Here's the drawing with two shaded views (mm, measured from the low corner). I have some questions. Give positions to 0.01 mm unless a question says otherwise; leave off trailing zeros. Loops run counter-clockwise (first coordinate to the right, second up) from the corner with the lowest first, then second, coordinate; pieces in that order, holes last. Notation, with made-up numbers: (-39.5, -38) -> (-19.5, -38) arc R18 cw to (-19.5, -16) -> close; hole circle Ø11 at (-30, -30). An arc over 180 degrees is marked (long way). Write each question's results on one line, items separated by ' | '. Start each with the question number.
Q1. If we section it at C-C, the plane y = 7.5: Give the number of separate pieces and of enclosed holes in the cut face, plus the area to 3 significant figures.
Q2. Will this pin go through, and if not, where does the flat tip stop? P1, Ø19, axis at x = 21, z = 35, coming from the +Y side.
Q3. If I drill on line 1 along X through (y, z) = (5, 5); line 2 along X through (y, z) = (5, 12.5) (1 decimal); line 3 along Y through (x, z) = (36, 7.25), over which ranges is the centre line in solid material (lowest first)?
Q4. If we section it at B-B, the plane z = 35: List the corners of the cut face in (x, y) for me, plus the area to 3 significant figures.
Q5. We'd pull the mould along Z, two halves only. Please class the marked faces 1, 2 and 3: released by +Z, released by -Z, zero draft, split by the parting line, or undercut.
Q6. If we section it at A-A, the plane x = 21: List the corners of the cut face in (y, z) for me.
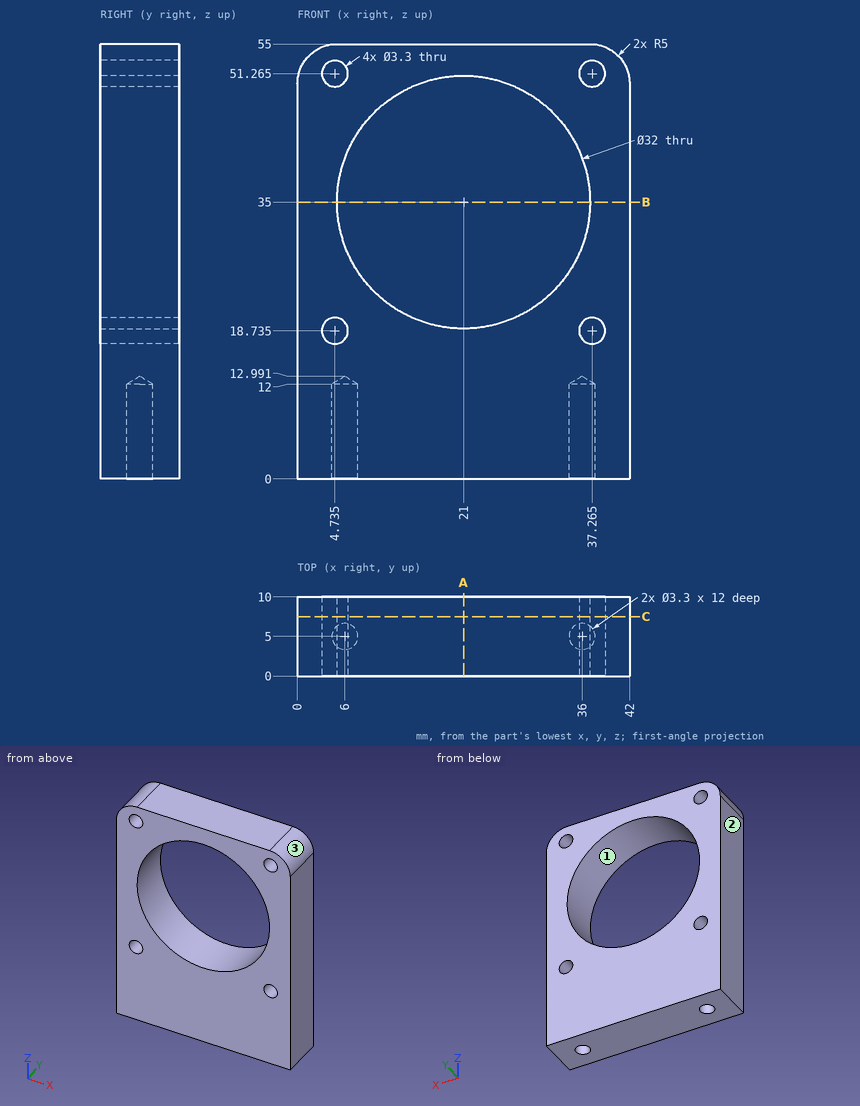
Final values:
1) separate pieces: 1 | enclosed holes: 5 | area: 1,460 mm²
2) P1: passes through
3) line 1: x = 0 to 4.35, 7.65 to 34.35, 37.65 to 42 | line 2: x = 0 to 5.2, 6.8 to 35.2, 36.8 to 42 | line 3: y = 0 to 3.35, 6.65 to 10
4) outline: (0, 0) -> (5, 0) -> (5, 10) -> (0, 10) -> close; (37, 0) -> (42, 0) -> (42, 10) -> (37, 10) -> close | area: 100 mm²
5) face 1: undercut | face 2: zero draft | face 3: released by +Z
6) outline: (0, 0) -> (10, 0) -> (10, 19) -> (0, 19) -> close; (0, 51) -> (10, 51) -> (10, 55) -> (0, 55) -> close
